Source: CAD feature listing. Evaluate the final solid. Frame: model axes, mm. Face numbers are marked on the shaded views. A direction names the side the tool comes from. Give positions to 0.01 mm unless a question says otherwise; leave off trailing zeros. Write each loop counter-clockwise with the first axis right and the second up, starting at its lowest first coordinate (ties: lowest second). Pieces come first, ordered by that corner, then holes. Notation, with made-up numbers: M 72,83 L 127,83 A14 cw 127,97 Z; hole C 74,45.5 d6. An arc over 180 degrees is marked long. Use CSV: the item, a comma, the result in double quotes. Start each with the question number.
from build123d import *

# Parameters (mm, degrees)
LEVER_BODY_41MM_DEPTH     = 20.5
PIVOT_EYE_BOSS_DEPTH      = 15.5
PIVOT_EYE_BOSS_DEPTH_BACK = 20.5
SKETCH1_4_R               = 9
EDGE_CHAMFER_3X45_A_SIZE  = 3
EDGE_CHAMFER_3X45_B_SIZE  = 3
UNDERSIDE_SLOT_SKETCH_W   = 12
UNDERSIDE_SLOT_SKETCH_H   = 7
UNDERSIDE_SLOT_DEPTH      = 145.5
TOP_HOLES_SKETCH_R        = 6
TOP_HOLES_2X_DEPTH        = 155.5


with BuildPart() as part:
    # Lever Profile Sketch → Lever Body 41mm (new, symmetric)
    with BuildSketch(Plane.XY):
        with BuildLine():
            Line((50, 21), (21, 21))
            Line((21, 21), (21, -21))
            Line((21, -21), (55, -21))
            ThreePointArc((55, -21), (62.071067812, -23.928932188), (65, -31))
            Line((65, -31), (65, -32.305162606))
            Line((65, -32.305162606), (110, -32.305162606))
            Line((110, -32.305162606), (110, -0.305162606))
            Line((110, -0.305162606), (64.918035459, -0.305162606))
            Line((64.918035459, -0.305162606), (50, 21))
        make_face()
    extrude(amount=LEVER_BODY_41MM_DEPTH, both=True)

    # Sketch1_4 → Pivot Eye Boss (add, two sides: drawn at the far end of the back side and taken through both)
    with BuildSketch(Plane.XY.offset(-PIVOT_EYE_BOSS_DEPTH_BACK)):
        with BuildLine():
            Line((21, 21), (0, 21))
            ThreePointArc((0, 21), (-21, 0), (0, -21))
            Line((0, -21), (21, -21))
            Line((21, -21), (21, 21))
        make_face()
        Circle(SKETCH1_4_R, mode=Mode.SUBTRACT)
    extrude(amount=PIVOT_EYE_BOSS_DEPTH + PIVOT_EYE_BOSS_DEPTH_BACK)

    # Edge Chamfer 3x45 A
    edge_chamfer_3x45_a_edges = [part.edges().sort_by_distance(p)[0] for p in [
        (35.5, 21, 20.5),
    ]]
    chamfer(edge_chamfer_3x45_a_edges, length=EDGE_CHAMFER_3X45_A_SIZE)

    # Edge Chamfer 3x45 B
    edge_chamfer_3x45_b_edges = [part.edges().sort_by_distance(p)[0] for p in [
        (110, -16.305162606, 20.5),
    ]]
    chamfer(edge_chamfer_3x45_b_edges, length=EDGE_CHAMFER_3X45_B_SIZE)

    # Underside Slot Sketch → Underside Slot (cut)
    with BuildSketch(Plane(origin=(110, 0, 0), x_dir=(0, 0, -1), z_dir=(1, 0, 0))):
        with Locations((0, -28.805162606)):
            Rectangle(UNDERSIDE_SLOT_SKETCH_W, UNDERSIDE_SLOT_SKETCH_H)
    extrude(amount=-UNDERSIDE_SLOT_DEPTH, mode=Mode.SUBTRACT)

    # Top Holes Sketch → Top Holes 2x (cut)
    with BuildSketch(Plane(origin=(0, 21, 0), x_dir=(1, 0, 0), z_dir=(0, 1, 0))):
        with Locations(Location((36, 0, 0), (0, 0, 270))):
            Circle(TOP_HOLES_SKETCH_R)
        with Locations(Location((86, 0, 0), (0, 0, 270))):
            Circle(TOP_HOLES_SKETCH_R)
    extrude(amount=-TOP_HOLES_2X_DEPTH, mode=Mode.SUBTRACT)


solid = part.part
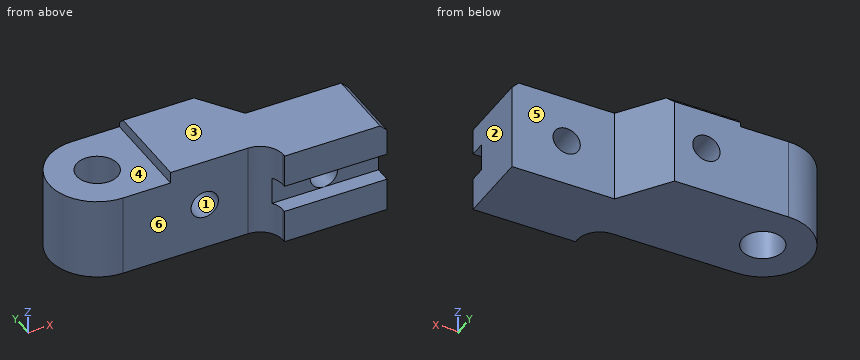
1. First-contact query: pin 1 (3 mm diameter, centred on x = 17, z = -2, fed in from -Y); pin 2 (1.5 mm diameter, centred on y = -5, z = 17.5, fed in from -X); pin 3 (5 mm diameter, centred on y = -1, z = -15.5, fed in from -X). Flat tips, straight axial feed; report the tip coordinate or a pass-through.
2. Access query for the marked faces 4, 5 and 6. Directions: +Z, -Z, +X, -X, +Y, -Y. A direction counts if a zero-diameter tool reaches every point of the face in a straight line with its end or side. Return the directions, or none.
3. Line query: probe 1 along Z at (x, y) = (86, -11); probe 2 along X at (y, z) = (2, 5.5); probe 3 along X at (y, z) = (-10, 0). Output: solid intervals per line, ascending.
4. Section A-A on z = 0. Return loops of the section in (x, y), then the cut area to 3 significant figures.
5. Section C-C on z = 11. Return loops of the section in (x, y).
6. Section B-B on y = -2.5. Return loops of the section in (x, z), then the cut area to 3 significant figures.
7. Pull-direction query (Z, two-part tool) for the marked faces 1, 2 and 3; classes: released by +Z, released by -Z, zero draft, split by the parting line, or undercut.
8. Section D-D on x = 36. Return loops of the section in (y, z), then the cut area to 3 significant figures.
Resolved:
1,pin 1,"stops at y = -21"
1,pin 2,"stops at x = 21"
1,pin 3,"stops at x = -21"
2,face 4,"+Z, -X, +Y, -Y"
2,face 5,"+Z, -Z, +X, +Y"
2,face 6,"+Z, -Z, -X, -Y"
3,probe 1,"z = -20.5 to -6, 6 to 20.5"
3,probe 2,"x = -20.9 to -8.77, 8.77 to 33.6, 38.4 to 63.3"
3,probe 3,"x = -18.47 to 30, 42 to 80, 92 to 110"
4,outline,"M 0,-21 L 30,-21 L 30,21 L 0,21 A21 ccw Z; M 42,-21 L 55,-21 A10 cw 63.22,-25.31 L 80,-25.31 L 80,-0.31 L 64.92,-0.31 L 50,21 L 42,21 Z; M 92,-25.31 L 110,-25.31 L 110,-0.31 L 92,-0.31 Z; hole C 0,0 d18"
4,area,"3,350 mm2"
5,outline,"M 0,-21 L 55,-21 A10 cw 65,-31 L 65,-32.31 L 110,-32.31 L 110,-0.31 L 64.92,-0.31 L 50,21 L 0,21 A21 ccw Z; hole C 0,0 d18"
6,outline,"M -20.85,-20.5 L -8.65,-20.5 L -8.65,15.5 L -20.85,15.5 Z; M 8.65,-20.5 L 110,-20.5 L 110,17.5 L 107,20.5 L 21,20.5 L 21,15.5 L 8.65,15.5 Z; hole C 36,0 d12; hole C 86,0 d12"
6,area,"4,300 mm2"
7,face 1,"undercut"
7,face 2,"zero draft"
7,face 3,"released by +Z"
8,outline,"M -21,-20.5 L 21,-20.5 L 21,-6 L -21,-6 Z; M -21,6 L 21,6 L 21,17.5 L 18,20.5 L -21,20.5 Z"
8,area,"1,210 mm2"
